```python
from build123d import *

# Parameters (mm, degrees)
SKETCH1_R                                           = 10
BOSS_EXTRUDE1_DEPTH                                 = 45
CBORE_FOR_M8_HEX_SOCKET_HEAD_CAP_SCREW1_D           = 9
CBORE_FOR_M8_HEX_SOCKET_HEAD_CAP_SCREW1_CBORE_D     = 15
CBORE_FOR_M8_HEX_SOCKET_HEAD_CAP_SCREW1_CBORE_DEPTH = 8.6
CHAMFER1_SIZE                                       = 0.5


with BuildPart() as part:
    # Sketch1 → Boss-Extrude1 (new body)
    with BuildSketch(Plane(origin=(0, 0, 0), x_dir=(1, 0, 0), z_dir=(0, 1, 0))):
        with Locations(Location((0, 0, 0), (0, 0, 90))):
            Circle(SKETCH1_R)
    extrude(amount=BOSS_EXTRUDE1_DEPTH)

    # CBORE for M8 Hex Socket Head Cap Screw1 (through all)
    with Locations(Plane(origin=(0, 45, 0), x_dir=(1, 0, 0), z_dir=(0, 1, 0))):
        with Locations((0, 0)):
            CounterBoreHole(CBORE_FOR_M8_HEX_SOCKET_HEAD_CAP_SCREW1_D / 2, CBORE_FOR_M8_HEX_SOCKET_HEAD_CAP_SCREW1_CBORE_D / 2, CBORE_FOR_M8_HEX_SOCKET_HEAD_CAP_SCREW1_CBORE_DEPTH)

    # Chamfer1
    chamfer1_edges = [part.edges().sort_by_distance(p)[0] for p in [
        (0, 0, 10),
        (0, 45, 10),
        (-7.5, 45, 0),
        (4.5, 0, 0),
    ]]
    chamfer(chamfer1_edges, length=CHAMFER1_SIZE)


solid = part.part
```
Model file for the job. Use its own axes, mm. A direction names the side the tool comes from. Coordinates: 2 decimals unless noted, no trailing zeros. Loops run counter-clockwise (first coordinate to the right, second up) from the corner with the lowest first, then second, coordinate; pieces in that order, holes last. Notation, with made-up numbers: (43.5, -20) -> (89.5, -20) arc R31 cw to (89.5, 11) -> close; hole circle Ø5 at (64, 4.25). An arc over 180 degrees is marked (long way). Answer as a JSON object with one key per item and string values.
Q1. Cut at A-A (z = 0). List the corners of the cut face in (x, y), and give its area (3 significant figures).
Report:
{"outline": "(-10, 0.5) -> (-9.5, 0) -> (-5, 0) -> (-4.5, 0.5) -> (-4.5, 36.4) -> (-7.5, 36.4) -> (-7.5, 44.5) -> (-8, 45) -> (-9.5, 45) -> (-10, 44.5) -> close; (4.5, 0.5) -> (5, 0) -> (9.5, 0) -> (10, 0.5) -> (10, 44.5) -> (9.5, 45) -> (8, 45) -> (7.5, 44.5) -> (7.5, 36.4) -> (4.5, 36.4) -> close", "area": "442 mm2"}
Q2. Probe probe 1 along X at (y, z) = (43, 0); probe 2 along X at (y, z) = (3, 0); probe 3 along Z at (x, y) = (-2.5, 20.5). List the from-to ranges inside material, lowest first.
Report:
{"probe 1": "x = -10 to -7.5, 7.5 to 10", "probe 2": "x = -10 to -4.5, 4.5 to 10", "probe 3": "z = -9.68 to -3.74, 3.74 to 9.68"}
Q3. Cut at C-C (y = 3). List the corners of the cut face in (x, z).
Report:
{"outline": "circle Ø20 at (0, 0); hole circle Ø9 at (0, 0)"}
Q4. Flat gauge pins, fed straight in: P1, Ø4.5, axis at x = 3.5, z = -1, coming from the +Y side; P2, Ø4, axis at y = 26.5, z = 5, coming from the -X side; P3, Ø8, axis at x = 5.5, y = 5.5, coming from the -Z side. Where does each tip first touch, or does it go through?
Report:
{"P1": "stops at y = 36.4", "P2": "stops at x = -9.54", "P3": "stops at z = -9.89"}
Q5. Pull direction X, two halves, no side cores. Call faces 1 (the flat face through (4, 0, -4)), 2 (the cylindrical face through (0.59, 18.2, -4.46)), 3 (the flat face through (0, 36.4, 5)), 4 (the cylindrical face through (9.76, 22.19, 2.17)): released by +X, released by -X, zero draft, split by the parting line, or undercut.
Report:
{"face 1": "zero draft", "face 2": "undercut", "face 3": "undercut", "face 4": "split by the parting line"}
Q6. 3-axis set-ups, long thin cutter, end or side, ignore diameter. For faces 5 (the cylindrical face through (-7.493, 40.507, -0.33)), 6 (the flat face through (7, 45, 4.3)): which of +Z, -Z, +X, -X, +Y, -Y reach the whole face in a straight line?
Report:
{"face 5": "+Y", "face 6": "+Z, -Z, +X, -X, +Y"}
Q7. Cut at B-B (x = 0). List the corners of the cut face in (y, z).
Report:
{"outline": "(0, -9.5) -> (0.5, -10) -> (44.5, -10) -> (45, -9.5) -> (45, -8) -> (44.5, -7.5) -> (36.4, -7.5) -> (36.4, -4.5) -> (0.5, -4.5) -> (0, -5) -> close; (0, 5) -> (0.5, 4.5) -> (36.4, 4.5) -> (36.4, 7.5) -> (44.5, 7.5) -> (45, 8) -> (45, 9.5) -> (44.5, 10) -> (0.5, 10) -> (0, 9.5) -> close"}
